from build123d import *

# Parameters (mm, degrees)
SKETCH_1_W          = 250
SKETCH_1_H          = 800
EXTRUDE_1_DEPTH     = 14
SKETCH_2_W          = 250
SKETCH_2_H          = 26
CUT_EXTRUDE_1_DEPTH = 1
CUT_EXTRUDE_2_REACH = 421.31
SKETCH_3_W          = 80
SKETCH_3_H          = 166.5
SKETCH_3_H_2        = 130
FILLET_1_R          = 10


with BuildPart() as part:
    # 草图1 → 凸台-拉伸1 (new body)
    with BuildSketch(Plane.XY):
        Rectangle(SKETCH_1_W, SKETCH_1_H)
    extrude(amount=EXTRUDE_1_DEPTH)

    # 草图2 → 切除-拉伸1 (cut)
    with BuildSketch(Plane.XY.offset(14)):
        with Locations((0, 187)):
            Rectangle(SKETCH_2_W, SKETCH_2_H)
        with Locations((0, 46)):
            Rectangle(SKETCH_2_W, SKETCH_2_H)
    extrude(amount=-CUT_EXTRUDE_1_DEPTH, mode=Mode.SUBTRACT)

    # 草图3 → 切除-拉伸2 (cut, up to next)
    with BuildSketch(Plane.XY.offset(14), mode=Mode.PRIVATE) as cut_extrude_2_sk1:
        with Locations((-55, -70.25)):
            Rectangle(SKETCH_3_W, SKETCH_3_H)
    cut_extrude_2_tool1 = extrude(cut_extrude_2_sk1.sketch, amount=-CUT_EXTRUDE_2_REACH, mode=Mode.PRIVATE) & part.part
    # 草图3 → 切除-拉伸2 (cut, up to next)
    with BuildSketch(Plane.XY.offset(14), mode=Mode.PRIVATE) as cut_extrude_2_sk2:
        with Locations((-55, -266.75)):
            Rectangle(SKETCH_3_W, SKETCH_3_H)
    cut_extrude_2_tool2 = extrude(cut_extrude_2_sk2.sketch, amount=-CUT_EXTRUDE_2_REACH, mode=Mode.PRIVATE) & part.part
    # 草图3 → 切除-拉伸2 (cut, up to next)
    with BuildSketch(Plane.XY.offset(14), mode=Mode.PRIVATE) as cut_extrude_2_sk3:
        with Locations((55, -266.75)):
            Rectangle(SKETCH_3_W, SKETCH_3_H)
    cut_extrude_2_tool3 = extrude(cut_extrude_2_sk3.sketch, amount=-CUT_EXTRUDE_2_REACH, mode=Mode.PRIVATE) & part.part
    # 草图3 → 切除-拉伸2 (cut, up to next)
    with BuildSketch(Plane.XY.offset(14), mode=Mode.PRIVATE) as cut_extrude_2_sk4:
        with Locations((55, -70.25)):
            Rectangle(SKETCH_3_W, SKETCH_3_H)
    cut_extrude_2_tool4 = extrude(cut_extrude_2_sk4.sketch, amount=-CUT_EXTRUDE_2_REACH, mode=Mode.PRIVATE) & part.part
    # 草图3 → 切除-拉伸2 (cut, up to next)
    with BuildSketch(Plane.XY.offset(14), mode=Mode.PRIVATE) as cut_extrude_2_sk5:
        with Locations((-55, 285)):
            Rectangle(SKETCH_3_W, SKETCH_3_H_2)
    cut_extrude_2_tool5 = extrude(cut_extrude_2_sk5.sketch, amount=-CUT_EXTRUDE_2_REACH, mode=Mode.PRIVATE) & part.part
    # 草图3 → 切除-拉伸2 (cut, up to next)
    with BuildSketch(Plane.XY.offset(14), mode=Mode.PRIVATE) as cut_extrude_2_sk6:
        with Locations((55, 285)):
            Rectangle(SKETCH_3_W, SKETCH_3_H_2)
    cut_extrude_2_tool6 = extrude(cut_extrude_2_sk6.sketch, amount=-CUT_EXTRUDE_2_REACH, mode=Mode.PRIVATE) & part.part
    add(cut_extrude_2_tool1.solids().sort_by_distance((-55, -70.25, 14))[0], mode=Mode.SUBTRACT)
    add(cut_extrude_2_tool2.solids().sort_by_distance((-55, -266.75, 14))[0], mode=Mode.SUBTRACT)
    add(cut_extrude_2_tool3.solids().sort_by_distance((55, -266.75, 14))[0], mode=Mode.SUBTRACT)
    add(cut_extrude_2_tool4.solids().sort_by_distance((55, -70.25, 14))[0], mode=Mode.SUBTRACT)
    add(cut_extrude_2_tool5.solids().sort_by_distance((-55, 285, 14))[0], mode=Mode.SUBTRACT)
    add(cut_extrude_2_tool6.solids().sort_by_distance((55, 285, 14))[0], mode=Mode.SUBTRACT)

    # 圆角1
    fillet_1_edges = [part.edges().sort_by_distance(p)[0] for p in [
        (-15, -183.5, 7),
        (-15, -350, 7),
        (-95, -350, 7),
        (-95, -183.5, 7),
        (95, -183.5, 7),
        (95, -350, 7),
        (15, -350, 7),
        (15, -183.5, 7),
        (95, 13, 7),
        (95, -153.5, 7),
        (15, -153.5, 7),
        (15, 13, 7),
        (-15, 350, 7),
        (-15, 220, 7),
        (-95, 220, 7),
        (-95, 350, 7),
        (95, 350, 7),
        (95, 220, 7),
        (15, 220, 7),
        (15, 350, 7),
        (-15, 13, 7),
        (-15, -153.5, 7),
        (-95, -153.5, 7),
        (-95, 13, 7),
    ]]
    fillet(fillet_1_edges, radius=FILLET_1_R)


solid = part.part
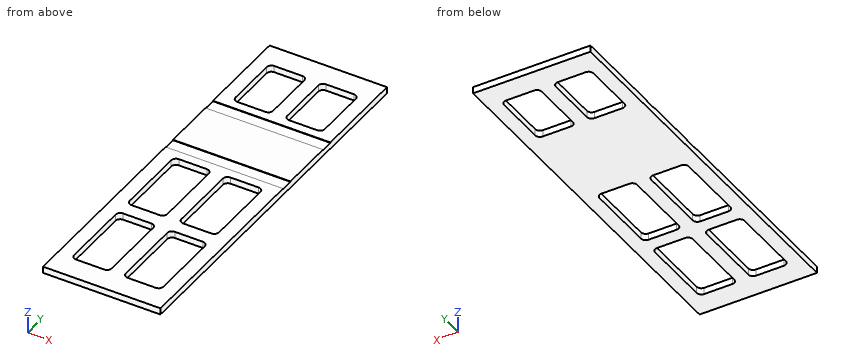
Build history of the part. All positions in model axes, mm. Round coordinates to 2 decimals unless told otherwise and drop trailing zeros. Write each loop counter-clockwise with the first axis right and the second up, starting at its lowest first coordinate (ties: lowest second). Pieces come first, ordered by that corner, then holes. Notation, with made-up numbers: M 67.5,15.5 L 88.5,15.5 A16 cw 88.5,37.5 Z; hole C 73.25,3.5 d1. An arc over 180 degrees is marked long. Use CSV: the item, a comma, the result in double quotes.
1. Saw through at D-D (y = 45). Give the cut face in (x, z).
Reply:
outline,"M -125,0 L 125,0 L 125,13 L -125,13 Z"
2. Saw through at C-C (z = 5.75). State how many separate pieces and enclosed holes the cut face has, plus the area to 3 significant figures.
Reply:
separate pieces,"1"
enclosed holes,"6"
area,"126,000 mm²"
3. Flat gauge pin, fed straight in: pin 1 (8 mm diameter, centred on x = 20.5, y = 183.5, fed in from +Z). Where does the tip first touch, or does it go through?
Reply:
pin 1,"stops at z = 13"
4. Saw through at B-B (y = 245). Give the cut face in (x, z).
Reply:
outline,"M -125,0 L -95,0 L -95,14 L -125,14 Z; M -15,0 L 15,0 L 15,14 L -15,14 Z; M 95,0 L 125,0 L 125,14 L 95,14 Z"
5. Saw through at A-A (x = 55). Give the cut face in (y, z), plus the area to 3 significant figures.
Reply:
outline,"M -400,0 L -350,0 L -350,14 L -400,14 Z; M -183.5,0 L -153.5,0 L -153.5,14 L -183.5,14 Z; M 13,0 L 220,0 L 220,14 L 200,14 L 200,13 L 174,13 L 174,14 L 59,14 L 59,13 L 33,13 L 33,14 L 13,14 Z; M 350,0 L 400,0 L 400,14 L 350,14 Z"
area,"4,670 mm²"
6. Wall check: probe 1 along X at (y, z) = (285.5, 9.5); probe 2 along Y at (x, z) = (35, 9.25); probe 3 along X at (y, z) = (229, 2.5). Give the ranges that are in metal, low to high. Write a range as from..to.
Reply:
probe 1,"x = -125..-95, -15..15, 95..125"
probe 2,"y = -400..-350, -183.5..-153.5, 13..220, 350..400"
probe 3,"x = -125..-94.95, -15.05..15.05, 94.95..125"
